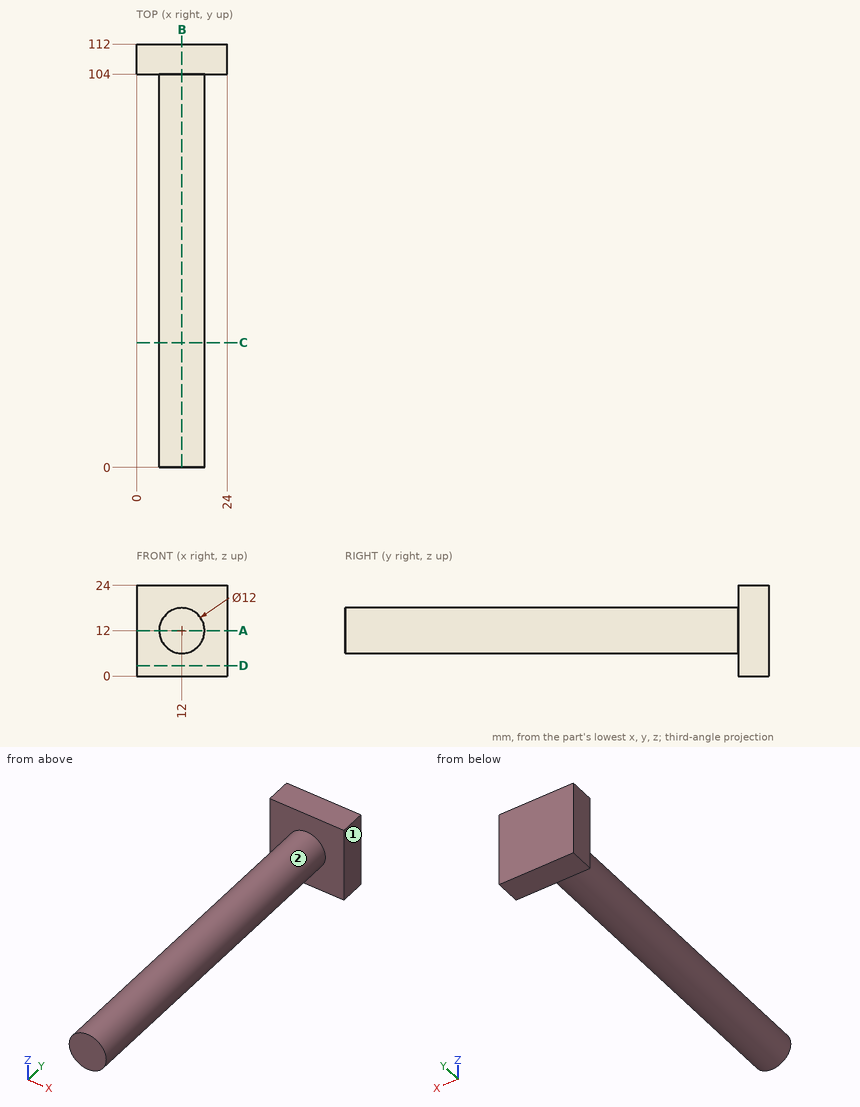
Here's the drawing with two shaded views (mm, measured from the low corner). I have some questions. A direction names the side the tool comes from. Round coordinates to 2 decimals unless told otherwise and drop trailing zeros. Loops run counter-clockwise (first coordinate to the right, second up) from the corner with the lowest first, then second, coordinate; pieces in that order, holes last.
Item 1: Which directions (+Z, -Z, +X, -X, +Y, -Y) give clear straight access to the entire face, cutting with the end or side of a thin tool? Please do the marked faces 1 and 2.
Item 2: Suppose I cut it at A-A, the plane z = 12. Write out the boundary of the cut face in (x, y), then the cut area to 3 significant figures.
Item 3: Will these pins go through, and if not, where does the flat tip stop? pin 1 Ø5 at (y, z) = (60.5, 7.5) entering from -X; pin 2 Ø8 at (y, z) = (65.5, 2.5) entering from +X; pin 3 Ø5 at (y, z) = (14.5, 12) entering from -X.
Item 4: Suppose I cut it at C-C, the plane y = 33. Write out the boundary of the cut face in (x, z).
Item 5: Suppose I cut it at B-B, the plane x = 12. Write out the boundary of the cut face in (y, z), then the cut area to 3 significant figures.
Item 6: Please list where these lines run through material, in increasing order: L1, parallel to Y at x = 18, z = 2.5; L2, parallel to Z at x = 12.5, y = 5; L3, parallel to X at y = 10, z = 15.25.
Item 7: Suppose I cut it at D-D, the plane z = 2.75. Write out the boundary of the cut face in (x, y).
Reported:
1. face 1: +Z, -Z, +X, +Y, -Y
1. face 2: -Y
2. outline: (0, 104) - (6, 104) - (6, 0) - (18, 0) - (18, 104) - (24, 104) - (24, 112) - (0, 112) - close
2. area: 1,440 mm2
3. pin 1: stops at x = 6.34
3. pin 2: stops at x = 14.4
3. pin 3: stops at x = 6
4. outline: circle Ø12 at (12, 12)
5. outline: (0, 6) - (104, 6) - (104, 0) - (112, 0) - (112, 24) - (104, 24) - (104, 18) - (0, 18) - close
5. area: 1,440 mm2
6. L1: y = 104 to 112
6. L2: z = 6.02 to 17.98
6. L3: x = 6.96 to 17.04
7. outline: (0, 104) - (24, 104) - (24, 112) - (0, 112) - close
